Part model, mm, in its own coordinate system. Face numbers are marked on the shaded views. Give positions to 0.01 mm unless a question says otherwise; leave off trailing zeros. Write each loop counter-clockwise with the first axis right and the second up, starting at its lowest first coordinate (ties: lowest second). Pieces come first, ordered by that corner, then holes.
from build123d import *


with BuildPart() as part:
    # 草图1 → 旋转1 (revolve)
    with BuildSketch(Plane(origin=(0, 0, 0), x_dir=(1, 0, 0), z_dir=(0, 1, 0)), mode=Mode.PRIVATE) as revolve_1_sk:
        Polygon((-15, 14.5), (-14.5, 15), (14.5, 15), (15, 14.5), (15, 12.75), (14.5, 12.25), (-14.5, 12.25), (-15, 12.75), align=None)
    revolve(revolve_1_sk.sketch.rotate(Axis((-1000, 0, 0), (1, 0, 0)), 180), axis=Axis((-1000, 0, 0), (1, 0, 0)))


solid = part.part
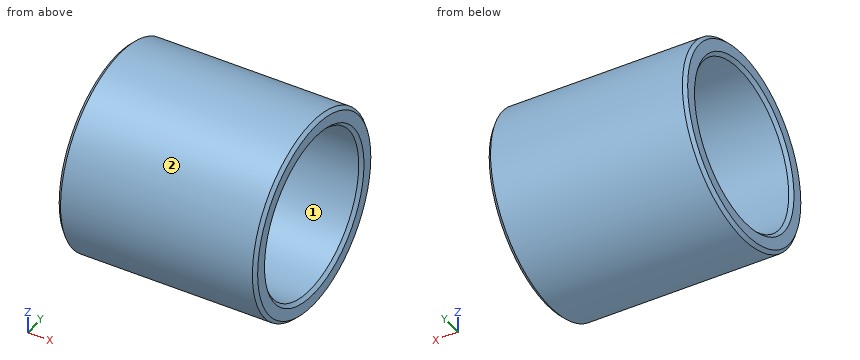
1) Saw through at C-C (x = -6.75). Write the cut outline in (y, z), and give its area (3 significant figures).
Check result:
outline: circle Ø30 at (0, 0); hole circle Ø24.5 at (0, 0)
area: 235 mm2
2) Mould opens along Y. For the marked faces 1 and 2 say: +Y half, -Y half, draft (parallel to the pull), parting line (faces both ways), or undercut.
Check result:
face 1: undercut
face 2: parting line
3) Flat gauge pins, fed straight in: P1, Ø5, axis at x = -10, y = -10, coming from the -Z side; P2, Ø5, axis at x = 8.5, y = -0.5, coming from the +Z side; P3, Ø6, axis at x = 1, z = 8, coming from the -Y side; P4, Ø8, axis at x = -9, y = -7, coming from the -Z side. Where does each tip first touch, or does it go through?
Check result:
P1: stops at z = -12.99
P2: stops at z = 15
P3: stops at y = -14.14
P4: stops at z = -14.7
4) Saw through at A-A (y = 0). Write the cut outline in (x, z), and give its area (3 significant figures).
Check result:
outline: (-15, -14.5) - (-14.5, -15) - (14.5, -15) - (15, -14.5) - (15, -12.75) - (14.5, -12.25) - (-14.5, -12.25) - (-15, -12.75) - close; (-15, 12.75) - (-14.5, 12.25) - (14.5, 12.25) - (15, 12.75) - (15, 14.5) - (14.5, 15) - (-14.5, 15) - (-15, 14.5) - close
area: 164 mm2
5) Drill centre lines: L1, parallel to Y at x = 8.5, z = 0; L2, parallel to Z at x = -1.25, y = -1.25; L3, parallel to Y at x = 13.75, z = 5. Where is each one in solid material? Low to high.
Check result:
L1: y = -15 to -12.25, 12.25 to 15
L2: z = -14.95 to -12.19, 12.19 to 14.95
L3: y = -14.14 to -11.18, 11.18 to 14.14
